Read the model definition and answer for the solid it produces. Units are mm, in the model's axes. A direction names the side the tool comes from. Give positions to 0.01 mm unless a question says otherwise; leave off trailing zeros. Loops run counter-clockwise (first coordinate to the right, second up) from the corner with the lowest first, then second, coordinate; pieces in that order, holes last. Notation, with made-up numbers: M 26,76 L 54,76 A11 cw 54,82 Z; hole C 17.5,47.5 d5. An arc over 180 degrees is marked long. Return JSON: item names as keys, results as strings. Group by question number.
```python
from build123d import *

# Parameters (mm, degrees)
SKETCH_2_R          = 10
SKETCH_2_W          = 10
SKETCH_2_H          = 10
CUT_EXTRUDE_1_DEPTH = 3


with BuildPart() as part:
    # 草图1 → 旋转1 (revolve)
    with BuildSketch(Plane(origin=(0, 0, 0), x_dir=(1, 0, 0), z_dir=(0, 1, 0)), mode=Mode.PRIVATE) as revolve_1_sk:
        Polygon((0, 54.5), (12.5, 54.5), (12.5, 39.5), (6, 39.5), (6, -20.5), (4, -20.5), (3.3235, -19.8235), (3.3235, -9.5), (0, -7.58117638), align=None)
    revolve(revolve_1_sk.sketch.rotate(Axis((0, 0, 20.5), (0, 0, -1)), 180), axis=Axis((0, 0, 20.5), (0, 0, -1)))

    # 草图2 → 切除-拉伸1 (cut)
    with BuildSketch(Plane.XY.offset(20.5)):
        Circle(SKETCH_2_R)
        Rectangle(SKETCH_2_W, SKETCH_2_H, mode=Mode.SUBTRACT)
    extrude(amount=-CUT_EXTRUDE_1_DEPTH, mode=Mode.SUBTRACT)


solid = part.part
```
1. For faces 4 (the flat face through (3, -5.4, -39.5)), 5 (the flat face through (0, -5, 19)), 6 (the flat face through (5, 0, 19)), 7 (the flat face through (-5, 0, 19)), 8 (the flat face through (0, 5, 19)), determine the directions among +Z, -Z, +X, -X, +Y, -Y from which every point of the face is accessible in a straight line to the end or side of a thin tool.
2. Find section C-C (y = -10.5). Write down the section's boundary in (x, z).
3. Find section D-D (z = -17). Write down the section's boundary in (x, y).
4. Flat-ended cylindrical pins translate along their axes: P1, Ø1.1, axis at x = -1.5, y = 5.5, coming from the +Z side; P2, Ø0.5, axis at x = 5.5, y = -1, coming from the +Z side; P3, Ø4, axis at x = 9.5, y = -6.5, coming from the +Z side; P4, Ø3.5, axis at y = -0.5, z = 19, coming from the +X side. Find the tip coordinate at first contact, or state that the pin passes through.
5. The mould has two halves that part along X. Classify faces 1 (the cylindrical face through (6, 0, -9)), 2 (the flat face through (0.1, 4.5, 20.5)), 3 (the cylindrical face through (-1.53, -2.95, 14.59)): +X half, -X half, draft (parallel to the pull), parting line (faces both ways), or undercut.
6. Straight lines are drawn through the part: line 1 along Y through (x, z) = (0, 15.25); line 2 along Z through (x, y) = (-3.5, 5.5); line 3 along Y through (x, z) = (-0.25, -42.5). For each, find the intervals that lie inside material, in ascending order.
7. Find section A-A (z = -40.5). Write down the section's boundary in (x, y).
8. Find section B-B (x = -9.25). Write down the section's boundary in (y, z).
Result:
{
 "1": {"face 4": "+Z", "face 5": "+Z, +X, -X, -Y", "face 6": "+Z, +X, +Y, -Y", "face 7": "+Z, -X, +Y, -Y", "face 8": "+Z, +X, -X, +Y"},
 "2": {"outline": "M -6.78,-54.5 L 6.78,-54.5 L 6.78,-39.5 L -6.78,-39.5 Z"},
 "3": {"outline": "C 0,0 d12"},
 "4": {"P1": "stops at z = 20.5", "P2": "stops at z = 17.5", "P3": "stops at z = -39.5", "P4": "stops at x = 6"},
 "5": {"face 1": "parting line", "face 2": "draft", "face 3": "undercut"},
 "6": {"line 1": "y = -6 to -3.32, 3.32 to 6", "line 2": "z = -54.5 to -39.5", "line 3": "y = -12.5 to 12.5"},
 "7": {"outline": "C 0,0 d25"},
 "8": {"outline": "M -8.41,-54.5 L 8.41,-54.5 L 8.41,-39.5 L -8.41,-39.5 Z"}
}
